from build123d import *

# Parameters (mm, degrees)
SKETCH_1_W          = 293
SKETCH_1_H          = 225
EXTRUDE_1_DEPTH     = 40
SKETCH_2_R          = 40
CUT_EXTRUDE_1_DEPTH = 25
SKETCH_3_R          = 28.7
CUT_EXTRUDE_2_DEPTH = 189.993386128
SKETCH_4_R          = 35
CUT_EXTRUDE_3_DEPTH = 189.993386128
SKETCH_5_R          = 31
CUT_EXTRUDE_4_DEPTH = 19.2
SKETCH_6_R          = 32.5
CUT_EXTRUDE_5_DEPTH = 2.2


with BuildPart() as part:
    # 草图1 → 凸台-拉伸1 (new body)
    with BuildSketch(Plane(origin=(0, 0, 0), x_dir=(1, 0, 0), z_dir=(0, 1, 0))):
        Rectangle(SKETCH_1_W, SKETCH_1_H)
    extrude(amount=EXTRUDE_1_DEPTH)

    # 草图2 → 切除-拉伸1 (cut)
    with BuildSketch(Plane.XZ):
        with Locations(Location((96.5, 0, 0), (0, 0, 270))):
            Circle(SKETCH_2_R)
    extrude(amount=-CUT_EXTRUDE_1_DEPTH, mode=Mode.SUBTRACT)

    # 草图3 → 切除-拉伸2 (cut, through all)
    with BuildSketch(Plane.XZ):
        with Locations(Location((-16, 0, 0), (0, 0, 270))):
            Circle(SKETCH_3_R)
    extrude(amount=-CUT_EXTRUDE_2_DEPTH, mode=Mode.SUBTRACT)

    # 草图4 → 切除-拉伸3 (cut, through all)
    with BuildSketch(Plane.XZ):
        with Locations(Location((96.5, 0, 0), (0, 0, 270))):
            Circle(SKETCH_4_R)
    extrude(amount=-CUT_EXTRUDE_3_DEPTH, mode=Mode.SUBTRACT)

    # 草图5 → 切除-拉伸4 (cut)
    with BuildSketch(Plane(origin=(0, 40, 0), x_dir=(1, 0, 0), z_dir=(0, 1, 0))):
        with Locations(Location((-16, 0, 0), (0, 0, 270))):
            Circle(SKETCH_5_R)
    extrude(amount=-CUT_EXTRUDE_4_DEPTH, mode=Mode.SUBTRACT)

    # 草图6 → 切除-拉伸5 (cut)
    with BuildSketch(Plane(origin=(0, 35, 0), x_dir=(1, 0, 0), z_dir=(0, 1, 0))):
        with Locations(Location((-16, 0, 0), (0, 0, 270))):
            Circle(SKETCH_6_R)
    extrude(amount=-CUT_EXTRUDE_5_DEPTH, mode=Mode.SUBTRACT)


solid = part.part
Work out the finished part from the listing and answer in its coordinate system (mm). A direction names the side the tool comes from. Give positions to 0.01 mm unless a question says otherwise; leave off trailing zeros. Write each loop counter-clockwise with the first axis right and the second up, starting at its lowest first coordinate (ties: lowest second). Pieces come first, ordered by that corner, then holes. Notation, with made-up numbers: (35.5, 54.25) - (42.5, 54.25) arc R8 ccw to (42.5, 63.25) - close; hole circle Ø3 at (-7, 24.25). An arc over 180 degrees is marked (long way). One line per item, written item: value. Start each with the question number.
1. For faces 4 (the flat face through (-25.04, 20.8, 27.41)), 5 (the flat face through (-28, 32.8, 29)), 6 (the flat face through (61, 25, 0)), determine the directions among +Z, -Z, +X, -X, +Y, -Y from which every point of the face is accessible in a straight line to the end or side of a thin tool.
2. Find section A-A (x = -16). Write down the section's boundary in (y, z).
3. Find section D-D (x = 96.5). Write down the section's boundary in (y, z), then the cut area to 3 significant figures.
4. Consider probe 1 along X at (y, z) = (32, 0); probe 2 along X at (y, z) = (33.8, 0); probe 3 along Z at (x, y) = (96, 19). Determine where each line is inside the solid, lowest interval first.
5. Find section B-B (y = 9). Write down the section's boundary in (x, z).
6. Find section C-C (z = 8.5). Write down the section's boundary in (x, y), then the cut area to 3 significant figures.
7. Given pin 1 (1 mm diameter, centred on x = 111, z = -50, fed in from -Y), flat-ended and moving along its own axis, determine where the tip first touches the part or whether it passes through.
8. For a pull along Y with two mould halves and no side action, classify faces 1 (the flat face through (-2, 20, 112.5)), 2 (the flat face through (-35, 40, -27)), 3 (the cylindrical face through (16.223, 33.915, -4.231)) as +Y half, -Y half, draft (parallel to the pull), parting line (faces both ways), or undercut.
Geometry results:
1. face 4: +Y
1. face 5: none
1. face 6: -Y
2. outline: (0, -112.5) - (40, -112.5) - (40, -31) - (35, -31) - (35, -32.5) - (32.8, -32.5) - (32.8, -31) - (20.8, -31) - (20.8, -28.7) - (0, -28.7) - close; (0, 28.7) - (20.8, 28.7) - (20.8, 31) - (32.8, 31) - (32.8, 32.5) - (35, 32.5) - (35, 31) - (40, 31) - (40, 112.5) - (0, 112.5) - close
3. outline: (0, -112.5) - (40, -112.5) - (40, -35) - (25, -35) - (25, -40) - (0, -40) - close; (0, 40) - (25, 40) - (25, 35) - (40, 35) - (40, 112.5) - (0, 112.5) - close
3. area: 5,950 mm2
4. probe 1: -146.5 to -47, 15 to 61.5, 131.5 to 146.5
4. probe 2: -146.5 to -48.5, 16.5 to 61.5, 131.5 to 146.5
4. probe 3: -112.5 to -40, 40 to 112.5
5. outline: (-146.5, -112.5) - (146.5, -112.5) - (146.5, 112.5) - (-146.5, 112.5) - close; hole circle Ø57.4 at (-16, 0); hole circle Ø80 at (96.5, 0)
6. outline: (-146.5, 0) - (-43.41, 0) - (-43.41, 20.8) - (-45.81, 20.8) - (-45.81, 32.8) - (-47.37, 32.8) - (-47.37, 35) - (-45.81, 35) - (-45.81, 40) - (-146.5, 40) - close; (11.41, 0) - (57.41, 0) - (57.41, 25) - (62.55, 25) - (62.55, 40) - (13.81, 40) - (13.81, 35) - (15.37, 35) - (15.37, 32.8) - (13.81, 32.8) - (13.81, 20.8) - (11.41, 20.8) - close; (130.45, 25) - (135.59, 25) - (135.59, 0) - (146.5, 0) - (146.5, 40) - (130.45, 40) - close
6. area: 6,460 mm2
7. pin 1: y = 0
8. face 1: draft
8. face 2: +Y half
8. face 3: undercut
